```python
from build123d import *

# Parameters (mm, degrees)
SKETCH1_R                = 4
BOSS_EXTRUDE1_DEPTH      = 3.5
SKETCH3_R                = 2.4
BOSS_EXTRUDE2_DEPTH      = 3.5
SKETCH2_R                = 1.5
CUT_EXTRUDE1_DEPTH       = 6
M2_5_TAPPED_HOLE1_REACH  = 13.358
M2_5_TAPPED_HOLE1_BORE_R = 1.025
CHAMFER1_SIZE            = 0.5
SKETCH6_OUTSIDE_W        = 12.66
SKETCH6_OUTSIDE_H        = 12.66
SKETCH6_OUTSIDE_W_2      = 11.194211724
SKETCH6_OUTSIDE_H_2      = 6.5
CUT_EXTRUDE2_DEPTH       = 10


with BuildPart() as part:
    # Sketch1 → Boss-Extrude1 (new body)
    with BuildSketch(Plane.XY):
        Circle(SKETCH1_R)
    extrude(amount=BOSS_EXTRUDE1_DEPTH)

    # Sketch3 → Boss-Extrude2 (add)
    with BuildSketch(Plane.XY.offset(3.5)):
        Circle(SKETCH3_R)
    extrude(amount=BOSS_EXTRUDE2_DEPTH)

    # Sketch2 → Cut-Extrude1 (cut)
    with BuildSketch(Plane(origin=(0, 0, 0), x_dir=(-1, 0, 0), z_dir=(0, 0, -1))):
        Circle(SKETCH2_R)
    extrude(amount=-CUT_EXTRUDE1_DEPTH, mode=Mode.SUBTRACT)

    # M2.5 Tapped Hole1 bore → M2.5 Tapped Hole1 (cut, up to next)
    with BuildSketch(Plane(origin=(4, 0, 0), x_dir=(0, 0, -1), z_dir=(1, 0, 0)), mode=Mode.PRIVATE) as m2_5_tapped_hole1_sk1:
        with Locations((-1.75, 0)):
            Circle(M2_5_TAPPED_HOLE1_BORE_R)
    m2_5_tapped_hole1_tool1 = extrude(m2_5_tapped_hole1_sk1.sketch, amount=-M2_5_TAPPED_HOLE1_REACH, mode=Mode.PRIVATE) & part.part
    add(m2_5_tapped_hole1_tool1.solids().sort_by_distance((4, 0, 1.75))[0], mode=Mode.SUBTRACT)

    # Chamfer1
    chamfer1_edges = [part.edges().sort_by_distance(p)[0] for p in [
        (-4, 0, 0),
        (-4, 0, 3.5),
        (-2.4, 0, 7),
    ]]
    chamfer(chamfer1_edges, length=CHAMFER1_SIZE)

    # Sketch6 outside → Cut-Extrude2 (cut)
    with BuildSketch(Plane.XY.offset(3.5)):
        Rectangle(SKETCH6_OUTSIDE_W, SKETCH6_OUTSIDE_H)
        Rectangle(SKETCH6_OUTSIDE_W_2, SKETCH6_OUTSIDE_H_2, mode=Mode.SUBTRACT)
    extrude(amount=-CUT_EXTRUDE2_DEPTH, mode=Mode.SUBTRACT)


solid = part.part
```
Here's how the part is built. I have some questions about the finished solid (model axes, mm). A direction names the side the tool comes from. Round coordinates to 2 decimals unless told otherwise and drop trailing zeros. Write each loop counter-clockwise with the first axis right and the second up, starting at its lowest first coordinate (ties: lowest second). Pieces come first, ordered by that corner, then holes. Notation, with made-up numbers: M 87.5,-33 L 110.5,-33 A12 ccw 110.5,-12 Z; hole C -6,3 d5. An arc over 180 degrees is marked long. Answer as CSV lines item,"result". Start each with the question number.
1. Suppose I cut it at C-C on z = 1.75. Write out the boundary of the cut face in (x, y) (3 decimals), then the cut area to 3 significant figures.
2. Suppose I cut it at D-D on z = 5.5. Write out the boundary of the cut face in (x, y), then the cut area to 3 significant figures.
3. Suppose I cut it at B-B on x = 0. Write out the boundary of the cut face in (y, z), then the cut area to 3 significant figures.
4. I'm going to push a flat-ended pin straight in: pin 1 Ø1 at (x, z) = (2, 4.5) entering from -Y. Where does the tip first touch, or does it pass through?
5. I need wall thicknesses on probe 1 along Y at (x, z) = (0, 4.75); probe 2 along Y at (x, z) = (1.9, 1.75) (3 decimals); probe 3 along X at (y, z) = (0, 2.25). Which ranges of each line are inside material? Lowest first, please.
6. Suppose I cut it at A-A on y = 0. Write out the boundary of the cut face in (x, z) (3 decimals), then the cut area to 3 significant figures.
7. On a 3-axis mill with a long thin cutter (end or side, diameter ignored), from which of +Z, -Z, +X, -X, +Y, -Y can I reach the whole of each face in a straight line? I mean faces 5 (the flat face through (-2, 0, 0)), 6 (the cylindrical face through (2.568, 0.308, 0.772)), 7 (the cylindrical face through (1.29, 2.024, 4.979)). Say none if no direction works.
8. Thinking about a two-plate mould opening in X: for faces 1 (the cylindrical face through (-4, 0, 2)), 2 (the flat face through (0, 0, 6)), 3 (the flat face through (0, -3.25, 2)), 4 (the cylindrical face through (-1.43, 0.45, 2.96)), which applies, released by +X, released by -X, zero draft, split by the parting line, or undercut?
Check result:
1,outline,"M -2.332,-3.25 L 2.332,-3.25 A4 ccw 3.866,-1.025 L 1.095,-1.025 A1.5 cw long 1.095,1.025 L 3.866,1.025 A4 ccw 2.332,3.25 L -2.332,3.25 A4 ccw Z"
1,area,"33.1 mm2"
2,outline,"C 0,0 d4.8; hole C 0,0 d3"
2,area,"11.0 mm2"
3,outline,"M -3.25,0 L -1.5,0 L -1.5,6 L 1.5,6 L 1.5,0 L 3.25,0 L 3.25,3.5 L 2.4,3.5 L 2.4,6.5 L 1.9,7 L -1.9,7 L -2.4,6.5 L -2.4,3.5 L -3.25,3.5 Z"
3,area,"21.3 mm2"
4,pin 1,"stops at y = -1.87"
5,probe 1,"y = -2.4 to -1.5, 1.5 to 2.4"
5,probe 2,"y = -3.25 to -1.025, 1.025 to 3.25"
5,probe 3,"x = -4 to -1.5"
6,outline,"M -4,0.5 L -3.5,0 L -1.5,0 L -1.5,6 L 1.5,6 L 1.5,2.775 L 4,2.775 L 4,3 L 3.5,3.5 L 2.4,3.5 L 2.4,6.5 L 1.9,7 L -1.9,7 L -2.4,6.5 L -2.4,3.5 L -3.5,3.5 L -4,3 Z; M 1.5,0 L 3.5,0 L 4,0.5 L 4,0.725 L 1.5,0.725 Z"
6,area,"20.9 mm2"
7,face 5,"-Z, +X, -X, +Y, -Y"
7,face 6,"+X"
7,face 7,"+Z"
8,face 1,"released by -X"
8,face 2,"undercut"
8,face 3,"zero draft"
8,face 4,"undercut"
